```python
from build123d import *

# Parameters (mm, degrees)
SKETCH1_W                    = 14
SKETCH1_H                    = 10.5
BOSS_EXTRUDE1_DEPTH          = 3
SKETCH2_W                    = 9.5
SKETCH2_H                    = 5
CUT_EXTRUDE1_DEPTH           = 2.5
CUT_EXTRUDE2_DEPTH           = 11.609547587
FILLET1_R                    = 1
SKETCH4_W                    = 3.8
SKETCH4_H                    = 5
CUT_EXTRUDE3_DEPTH           = 11.609547587
M2_5_TAPPED_HOLE1_D          = 2.05
F_1_0_1_DIAMETER_HOLE1_D     = 1
F_2_0_2_DIAMETER_HOLE1_D     = 2
CUT_EXTRUDE4_DEPTH           = 11.609547587
F_3_0_3_DIAMETER_HOLE1_D     = 3
F_3_0_3_DIAMETER_HOLE1_DEPTH = 4
F_3_0_3_DIAMETER_HOLE1_TIP   = 0.901290929
FILLET2_R                    = 0.5
M2_5_TAPPED_HOLE2_D          = 2.05
M2_5_TAPPED_HOLE2_DEPTH      = 4
M2_5_TAPPED_HOLE2_TIP        = 0.615882135


with BuildPart() as part:
    # Sketch1 → Boss-Extrude1 (new, symmetric)
    with BuildSketch(Plane.XY):
        Rectangle(SKETCH1_W, SKETCH1_H)
    extrude(amount=BOSS_EXTRUDE1_DEPTH, both=True)

    # Sketch2 → Cut-Extrude1 (cut)
    with BuildSketch(Plane.XY.offset(3)):
        with Locations((2.25, 2.75)):
            Rectangle(SKETCH2_W, SKETCH2_H)
    extrude(amount=-CUT_EXTRUDE1_DEPTH, mode=Mode.SUBTRACT)

    # Sketch3 → Cut-Extrude2 (cut, through all)
    with BuildSketch(Plane.XY.offset(3)):
        Polygon((-7, 5.25), (-1, 5.25), (-1, 3.25), (-7, 2.25), align=None)
    extrude(amount=-CUT_EXTRUDE2_DEPTH, mode=Mode.SUBTRACT)

    # Fillet1
    fillet1_edges = [part.edges().sort_by_distance(p)[0] for p in [
        (-2.5, 0.25, 1.75),
        (-1, 3.25, -1.25),
    ]]
    fillet(fillet1_edges, radius=FILLET1_R)

    # Sketch4 → Cut-Extrude3 (cut, through all)
    with BuildSketch(Plane.XY.offset(3)):
        with Locations((-5.1, -1.25)):
            Rectangle(SKETCH4_W, SKETCH4_H)
    extrude(amount=-CUT_EXTRUDE3_DEPTH, mode=Mode.SUBTRACT)

    # M2.5 Tapped Hole1 (through all)
    with Locations(Plane.XY.offset(0.5)):
        with Locations((3, 2.75)):
            Hole(M2_5_TAPPED_HOLE1_D / 2)

    # Ø1.0 (1) Diameter Hole1 (through all)
    with Locations(Plane.XY.offset(0.5)):
        with Locations((0, 2.75), (6, 2.75)):
            Hole(F_1_0_1_DIAMETER_HOLE1_D / 2)

    # Ø2.0 (2) Diameter Hole1 (through all)
    with Locations(Plane.XY.offset(3)):
        with Locations((-1, -1.75)):
            Hole(F_2_0_2_DIAMETER_HOLE1_D / 2)

    # Sketch15 → Cut-Extrude4 (cut, through all)
    with BuildSketch(Plane.XY.offset(3)):
        Polygon((7, -5.25), (1, -5.25), (1.7, -4.55), (7, -4.55), align=None)
    extrude(amount=-CUT_EXTRUDE4_DEPTH, mode=Mode.SUBTRACT)

    # Ø3.0 (3) Diameter Hole1
    with Locations(Plane(origin=(0, -4.55, 0), x_dir=(-1, 0, 0), z_dir=(0, -1, 0))):
        with Locations((-4.2, 0)):
            Hole(F_3_0_3_DIAMETER_HOLE1_D / 2, depth=F_3_0_3_DIAMETER_HOLE1_DEPTH)
            with Locations((0, 0, -(F_3_0_3_DIAMETER_HOLE1_DEPTH + F_3_0_3_DIAMETER_HOLE1_TIP / 2))):  # 118° drill point
                Cone(0, F_3_0_3_DIAMETER_HOLE1_D / 2, F_3_0_3_DIAMETER_HOLE1_TIP, mode=Mode.SUBTRACT)

    # Fillet2
    fillet2_edges = [part.edges().sort_by_distance(p)[0] for p in [
        (-7, -3.75, 0),
        (-7, 1.25, 0),
    ]]
    fillet(fillet2_edges, radius=FILLET2_R)

    # M2.5 Tapped Hole2
    with Locations(Plane(origin=(0, -5.25, 0), x_dir=(-1, 0, 0), z_dir=(0, -1, 0))):
        with Locations((1, 0)):
            Hole(M2_5_TAPPED_HOLE2_D / 2, depth=M2_5_TAPPED_HOLE2_DEPTH)
            with Locations((0, 0, -(M2_5_TAPPED_HOLE2_DEPTH + M2_5_TAPPED_HOLE2_TIP / 2))):  # 118° drill point
                Cone(0, M2_5_TAPPED_HOLE2_D / 2, M2_5_TAPPED_HOLE2_TIP, mode=Mode.SUBTRACT)


solid = part.part
```
Work out the finished part from the listing and answer in its coordinate system (mm). A direction names the side the tool comes from. Give positions to 0.01 mm unless a question says otherwise; leave off trailing zeros. Order: outer loops, then holes, each group sorted by start corner. A loop starts at its lowest first (then second) coordinate and runs counter-clockwise, first axis right, second up. Notation, with made-up numbers: M 9,58.25 L 59,58.25 A30 ccw 59,88.25 Z; hole C -32,-10 d4. An arc over 180 degrees is marked long. Return JSON: item names as keys, results as strings.
1) Section C-C, the plane y = 2.75 is taken. Write down the section's boundary in (x, z) (3 decimals).
Resolved:
{"outline": "M -4,-3 L -0.5,-3 L -0.5,0.5 L -2.5,0.5 L -2.5,3 L -4,3 Z; M 0.5,-3 L 1.975,-3 L 1.975,0.5 L 0.5,0.5 Z; M 4.025,-3 L 5.5,-3 L 5.5,0.5 L 4.025,0.5 Z; M 6.5,-3 L 7,-3 L 7,0.5 L 6.5,0.5 Z"}
2) Straight lines are drawn through the part: line 1 along X through (y, z) = (-1, 0.25); line 2 along Z through (x, y) = (4.2, -2.05); line 3 along X through (y, z) = (4.25, -1). For each, find the intervals that lie inside material, in ascending order. Write a range as [from, to].
Resolved:
{"line 1": "[-3.2, -1.66], [-0.34, 2.72], [5.68, 7]", "line 2": "[-3, -1.5], [1.5, 3]", "line 3": "[-1, 7]"}
3) Section A-A, the plane y = -1.75 is taken. Write down the section's boundary in (x, z) (3 decimals), plus the area to 3 significant figures.
Resolved:
{"outline": "M -3.2,-3 L -2,-3 L -2,-0.225 A1.025 cw -2,0.225 L -2,3 L -3.2,3 Z; M 0,-3 L 7,-3 L 7,3 L 0,3 L 0,0.225 A1.025 cw 0,-0.225 Z; hole C 4.2,0 d3", "area": "42.1 mm^2"}
4) A tool of negligible diameter and unlimited length cuts with its end or side. For faces 1 (the cylindrical face through (-2.024, -3.666, -0.045)), 2 (the flat face through (-3.2, -1, 0)), 3 (the flat face through (-1, 5, -1)), from which of +Z, -Z, +X, -X, +Y, -Y can it reach the whole face along a straight path? Write none if from no direction.
Resolved:
{"face 1": "-Y", "face 2": "+Z, -Z, -X", "face 3": "+Z, -Z, -X, +Y"}
5) Section D-D, the plane x = -5.25 is taken. Write down the section's boundary in (y, z).
Resolved:
{"outline": "M -5.25,-3 L -3.75,-3 L -3.75,3 L -5.25,3 Z; M 1.25,-3 L 2.54,-3 L 2.54,3 L 1.25,3 Z"}
6) For a pull along Y with two mould halves and no side action, classify faces 4 (the flat face through (1, -2, 3)), 5 (the flat face through (5.5, -4.55, 1.4)), 6 (the cylindrical face through (0.065, 3.246, -1.274)) as +Y half, -Y half, draft (parallel to the pull), parting line (faces both ways), or undercut.
Resolved:
{"face 4": "draft", "face 5": "-Y half", "face 6": "undercut"}
7) Section B-B, the plane z = -1.75 is taken. Write down the section's boundary in (x, y) (3 decimals).
Resolved:
{"outline": "M -7,-5.25 L 1,-5.25 L 1.7,-4.55 L 7,-4.55 L 7,5.25 L -1,5.25 L -1,4.097 A1 cw -1.836,3.111 L -7,2.25 L -7,1.75 A0.5 ccw -6.5,1.25 L -3.2,1.25 L -3.2,-3.75 L -6.5,-3.75 A0.5 ccw -7,-4.25 Z; hole C -1,-1.75 d2; hole C 0,2.75 d1; hole C 3,2.75 d2.05; hole C 6,2.75 d1"}
8) Each of these flat-tipped pins is pushed along its axis until it touches: pin 1 (1.3 mm diameter, centred on y = 4.5, z = -1, fed in from -X); pin 2 (2.5 mm diameter, centred on x = 4, z = 1, fed in from -Y); pin 3 (1.6 mm diameter, centred on x = -5.5, z = -1.5, fed in from +Y). Where does it stop, or does it pass through?
Resolved:
{"pin 1": "x = -1.03", "pin 2": "y = -4.55", "pin 3": "y = 2.63"}
